```python
from build123d import *

# Parameters (mm, degrees)
SKETCH_1_W                = 400
SKETCH_1_H                = 150
EXTRUDE_1_DEPTH           = 15
HOLE_WIZARD_1_D           = 9
HOLE_WIZARD_1_CBORE_D     = 15
HOLE_WIZARD_1_CBORE_DEPTH = 9


with BuildPart() as part:
    # 草图1 → 凸台-拉伸1 (new body)
    with BuildSketch(Plane(origin=(0, 0, 0), x_dir=(0, 0, -1), z_dir=(1, 0, 0))):
        Rectangle(SKETCH_1_W, SKETCH_1_H)
    extrude(amount=EXTRUDE_1_DEPTH)

    # 打孔尺寸(%根据)内六角圆柱头螺钉的类型1 (through all)
    with Locations(Plane(origin=(15, 0, 0), x_dir=(0, 0, -1), z_dir=(1, 0, 0))):
        with Locations((-150, 50), (0, 50), (150, 50), (-150, -50), (0, -50), (150, -50)):
            CounterBoreHole(HOLE_WIZARD_1_D / 2, HOLE_WIZARD_1_CBORE_D / 2, HOLE_WIZARD_1_CBORE_DEPTH)


solid = part.part
```
For this review, take the finished solid that the model builds, in its own axes (mm). A direction names the side the tool comes from. Round coordinates to 2 decimals unless told otherwise and drop trailing zeros. Loops run counter-clockwise (first coordinate to the right, second up) from the corner with the lowest first, then second, coordinate; pieces in that order, holes last.
Q1. Add section A-A on z = 150. Write out the cut boundary in (x, y), plus the area to 3 significant figures.
Result sheet:
outline: (0, -75) - (15, -75) - (15, -57.5) - (6, -57.5) - (6, -54.5) - (0, -54.5) - close; (0, -45.5) - (6, -45.5) - (6, -42.5) - (15, -42.5) - (15, 42.5) - (6, 42.5) - (6, 45.5) - (0, 45.5) - close; (0, 54.5) - (6, 54.5) - (6, 57.5) - (15, 57.5) - (15, 75) - (0, 75) - close
area: 1,870 mm2
Q2. Insertion check: pin 1 Ø7.5 at (y, z) = (51.5, -149) entering from +X. The pin has a flat end and moves straight along its axis. Give the tip position at first contact, or say it passes through.
Result sheet:
pin 1: stops at x = 6
Q3. Mouldability with a two-part tool opening along Y and no side actions: class faces 3 (the face through (7, 75, 3)), 4 (the face through (0, 1, 3)), 5 (the face through (7, -75, 3)), 6 (the face through (6, 50, 145)) as +Y half, -Y half, draft (parallel to the pull), parting line (faces both ways), or undercut.
Result sheet:
face 3: +Y half
face 4: draft
face 5: -Y half
face 6: undercut
Q4. Add section C-C on x = 12.25. Write out the cut boundary in (y, z).
Result sheet:
outline: (-75, -200) - (75, -200) - (75, 200) - (-75, 200) - close; hole circle Ø15 at (-50, -150); hole circle Ø15 at (-50, 0); hole circle Ø15 at (-50, 150); hole circle Ø15 at (50, -150); hole circle Ø15 at (50, 0); hole circle Ø15 at (50, 150)
Q5. Machinability: for faces 1 (the face through (6, 45, 0)), 2 (the face through (2.96, 46.01, -147.92)), which of the approach directions +Z, -Z, +X, -X, +Y, -Y give a long, thin tool a straight path to every point of the face, cutting with its end or side? Answer none if there is none.
Result sheet:
face 1: +X
face 2: +X, -X
Q6. Add section B-B on y = 50. Write out the cut boundary in (x, z), plus the area to 3 significant figures.
Result sheet:
outline: (0, -200) - (15, -200) - (15, -157.5) - (6, -157.5) - (6, -154.5) - (0, -154.5) - close; (0, -145.5) - (6, -145.5) - (6, -142.5) - (15, -142.5) - (15, -7.5) - (6, -7.5) - (6, -4.5) - (0, -4.5) - close; (0, 4.5) - (6, 4.5) - (6, 7.5) - (15, 7.5) - (15, 142.5) - (6, 142.5) - (6, 145.5) - (0, 145.5) - close; (0, 154.5) - (6, 154.5) - (6, 157.5) - (15, 157.5) - (15, 200) - (0, 200) - close
area: 5,430 mm2
Q7. To check wall thickness, follow line 1 along Y through (x, z) = (8, -146); line 2 along Y through (x, z) = (8.5, -150); line 3 along Z through (x, y) = (12.25, -45.5). State the ranges of each line that lie inside material, in increasing order.
Result sheet:
line 1: y = -75 to -56.34, -43.66 to 43.66, 56.34 to 75
line 2: y = -75 to -57.5, -42.5 to 42.5, 57.5 to 75
line 3: z = -200 to -156, -144 to -6, 6 to 144, 156 to 200
